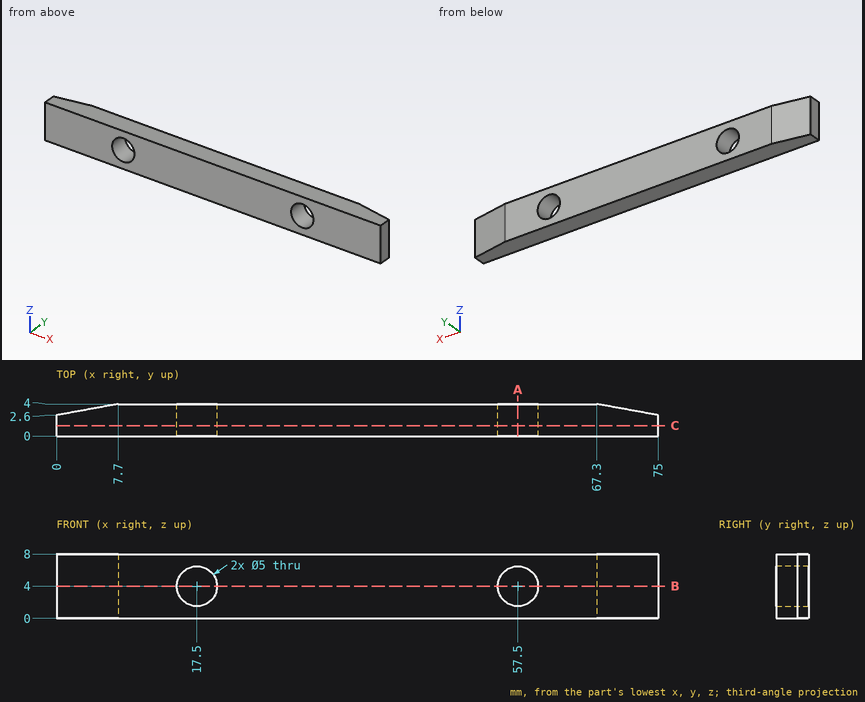
Geometry check sheet. Reference: drawing and pictorial views, mm from the part's lowest x, y, z. Give positions to 0.01 mm unless a question says otherwise; leave off trailing zeros. Loops run counter-clockwise (first coordinate to the right, second up) from the corner with the lowest first, then second, coordinate; pieces in that order, holes last. Notation, with made-up numbers: (76.5, 10) - (92.5, 10) arc R25 ccw to (92.5, 40) - close; hole circle Ø3 at (29.5, 18). An arc over 180 degrees is marked (long way). One line per question, with ' | ' between items. Start each with the question number.
1. Cross-section at A-A, the plane x = 57.5. Enter the section's corners in (y, z).
2. Gauge pin test, flat ends, axial feed: pin 1 Ø1 at (x, z) = (18, 5) entering from +Y; pin 2 Ø4 at (x, z) = (32, 3) entering from -Y. Record the tip position at first contact, or that the pin passes through.
3. Cross-section at C-C, the plane y = 1.3. Enter the section's corners in (x, z), plus the area to 3 significant figures.
4. Material ranges on line 1 along X through (y, z) = (2.05, 4); line 2 along X through (y, z) = (1.95, 5.5); line 3 along Y through (x, z) = (4.5, 1.5), recorded low to high. Write a range as [from, to].
5. Cross-section at B-B, the plane z = 4. Enter the section's corners in (x, y), plus the area to 3 significant figures.
Check result:
1) outline: (0, 0) - (4, 0) - (4, 1.5) - (0, 1.5) - close; (0, 6.5) - (4, 6.5) - (4, 8) - (0, 8) - close
2) pin 1: passes through | pin 2: stops at y = 0
3) outline: (0, 0) - (75, 0) - (75, 8) - (0, 8) - close; hole circle Ø5 at (17.5, 4); hole circle Ø5 at (57.5, 4) | area: 561 mm2
4) line 1: x = [0, 15], [20, 55], [60, 75] | line 2: x = [0, 15.5], [19.5, 55.5], [59.5, 75] | line 3: y = [0, 3.42]
5) outline: (0, 0) - (15, 0) - (15, 4) - (7.7, 4) - (0, 2.6) - close; (20, 0) - (55, 0) - (55, 4) - (20, 4) - close; (60, 0) - (75, 0) - (75, 2.6) - (67.3, 4) - (60, 4) - close | area: 249 mm2
